The listing builds one solid part. Answer for the finished solid, in the listing's coordinates (mm). A direction names the side the tool comes from. Round coordinates to 2 decimals unless told otherwise and drop trailing zeros. Order: outer loops, then holes, each group sorted by start corner. A loop starts at its lowest first (then second) coordinate and runs counter-clockwise, first axis right, second up. Notation, with made-up numbers: (-6, 78) - (15, 78) arc R29 cw to (15, 105) - close; hole circle Ø11 at (-39.75, 57.25). An arc over 180 degrees is marked (long way). One line per item, written item: value. Start each with the question number.
1. Section C-C, the plane y = -8.5 is taken. Give the vertices of the cut face in (x, z).
2. Section D-D, the plane x = 5.5 is taken. Give the vertices of the cut face in (y, z), then the cut area to 3 significant figures.
3. A tool of negligible diameter and unlimited length cuts with its end or side. For faces 4 (the flat face through (0.74, 4.573, 0.084)), 5 (the flat face through (30, 24, 0)), 6 (the flat face through (68, 3, 0)), 7 (the flat face through (2, 11, 0)), from which of +Z, -Z, +X, -X, +Y, -Y can it reach the whole face along a straight path? Write none if from no direction.
4. Section A-A, the plane x = 27 is taken. Give the vertices of the cut face in (y, z).
5. Section B-B, the plane z = -0.5 is taken. Give the vertices of the cut face in (x, y).
6. Straight lines are drawn through the part: line 1 (Y direction, x = 3, z = 3.5); line 2 (X direction, y = 8, z = -4.5); line 3 (X direction, y = -3, z = 2). For each, find the intervals that lie inside material, in ascending order.
7. Flat-ended cylindrical pins translate along their axes: P1, Ø0.6, axis at x = 12, z = 0, coming from the +Y side; P2, Ø4, axis at y = 7.5, z = -2, coming from the -X side; P3, Ø1.2, axis at y = -1, z = 1.5, coming from the -X side. Find the tip coordinate at first contact, or state that the pin passes through.
8. For a pull along Y with two mould halves and no side action, classify faces 1 (the flat face through (24, -17, 0)), 2 (the flat face through (4.5, 8, 0)), 3 (the flat face through (36, -12.5, 0)) as released by +Y, released by -Y, zero draft, split by the parting line, or undercut.
from build123d import *

# Parameters (mm, degrees)
EXTRUDE_1_DEPTH     = 6
CUT_EXTRUDE_1_DEPTH = 64.442887702
SKETCH_3_W          = 60
SKETCH_3_H          = 4
CUT_EXTRUDE_2_DEPTH = 1
CHAMFER_1_SIZE      = 1


with BuildPart() as part:
    # 草图1 → 凸台-拉伸1 (new, symmetric)
    with BuildSketch(Plane.XY):
        with BuildLine():
            Line((0, 0), (0, 5))
            Line((0, 5), (1.5, 4.133974596))
            ThreePointArc((1.5, 4.133974596), (3.5, 4.133974596), (4.5, 5.866025404))
            Line((4.5, 5.866025404), (4.5, 9.5))
            ThreePointArc((4.5, 9.5), (4.060660172, 10.560660172), (3, 11))
            Line((3, 11), (0, 11))
            Line((0, 11), (0, 25))
            Line((0, 25), (60, 25))
            Line((60, 25), (60, 1))
            Line((60, 1), (64, 1))
            Line((64, 1), (66, 3))
            Line((66, 3), (70, 3))
            Line((70, 3), (70, -12.5))
            Line((70, -12.5), (60, -12.5))
            Line((60, -12.5), (60, -21.552558883))
            Line((60, -21.552558883), (49, -24.5))
            Line((49, -24.5), (48, -24.5))
            Line((48, -24.5), (48, -12.5))
            Line((48, -12.5), (24, -12.5))
            Line((24, -12.5), (24, -21.552558883))
            Line((24, -21.552558883), (13, -24.5))
            Line((13, -24.5), (12, -24.5))
            Line((12, -24.5), (12, -1.5))
            Line((12, -1.5), (12.5, -1.5))
            Line((12.5, -1.5), (12.5, 0))
            Line((12.5, 0), (0, 0))
        make_face()
    extrude(amount=EXTRUDE_1_DEPTH, both=True)

    # 草图2 → 切除-拉伸1 (cut, through all)
    with BuildSketch(Plane.ZY.offset(-12)):
        Polygon((6, -17.57179677), (6, -29.5), (-6, -29.5), (-6, -17.57179677), (-2, -24.5), (2, -24.5), align=None)
    extrude(amount=-CUT_EXTRUDE_1_DEPTH, mode=Mode.SUBTRACT)

    # 草图3 → 切除-拉伸2 (cut)
    with BuildSketch(Plane(origin=(0, 25, 0), x_dir=(1, 0, 0), z_dir=(0, 1, 0))):
        with Locations((30, 0)):
            Rectangle(SKETCH_3_W, SKETCH_3_H)
    extrude(amount=-CUT_EXTRUDE_2_DEPTH, mode=Mode.SUBTRACT)

    # 倒角1
    chamfer_1_edges = [part.edges().sort_by_distance(p)[0] for p in [
        (70, -4.75, -6),
        (70, -4.75, 6),
    ]]
    chamfer(chamfer_1_edges, length=CHAMFER_1_SIZE)


solid = part.part
Answer list:
1. outline: (12, -6) - (69, -6) - (70, -5) - (70, 5) - (69, 6) - (12, 6) - close
2. outline: (0, -6) - (25, -6) - (25, -2) - (24, -2) - (24, 2) - (25, 2) - (25, 6) - (0, 6) - close
2. area: 296 mm²
3. face 4: +Z, -Z
3. face 5: +X, -X, +Y
3. face 6: +Z, -Z, +X, +Y
3. face 7: +Z, -Z, -X
4. outline: (-12.5, -6) - (25, -6) - (25, -2) - (24, -2) - (24, 2) - (25, 2) - (25, 6) - (-12.5, 6) - close
5. outline: (0, 0) - (12.5, 0) - (12.5, -1.5) - (12, -1.5) - (12, -24.5) - (13, -24.5) - (24, -21.55) - (24, -12.5) - (48, -12.5) - (48, -24.5) - (49, -24.5) - (60, -21.55) - (60, -12.5) - (70, -12.5) - (70, 3) - (66, 3) - (64, 1) - (60, 1) - (60, 24) - (0, 24) - (0, 11) - (3, 11) arc R1.5 cw to (4.5, 9.5) - (4.5, 5.87) arc R2 cw to (1.5, 4.13) - (0, 5) - close
6. line 1: y = 0 to 3.93, 11 to 25
6. line 2: x = 4.5 to 60
6. line 3: x = 12 to 70
7. P1: stops at y = 24
7. P2: stops at x = 4.47
7. P3: stops at x = 12
8. face 1: zero draft
8. face 2: undercut
8. face 3: released by -Y
